```python
from build123d import *

# Parameters (mm, degrees)
BOSS_EXTRUDE1_DEPTH    = 11
SKETCH2_R              = 13
BOSS_EXTRUDE2_DEPTH    = 1
SKETCH3_R              = 9.5
CUT_EXTRUDE1_DEPTH     = 25.372115214
M5_TAPPED_HOLE1_REACH  = 37.623
M5_TAPPED_HOLE1_BORE_R = 2.1
M5_TAPPED_HOLE2_REACH  = 37.623
M5_TAPPED_HOLE2_BORE_R = 2.1


with BuildPart() as part:
    # Sketch1 → Boss-Extrude1 (new body)
    with BuildSketch(Plane.XY):
        with BuildLine():
            Line((-9.013878189, 15), (9.013878189, 15))
            ThreePointArc((9.013878189, 15), (12.374368671, 12.374368671), (15, 9.013878189))
            Line((15, 9.013878189), (15, -9.013878189))
            ThreePointArc((15, -9.013878189), (12.374368671, -12.374368671), (9.013878189, -15))
            Line((9.013878189, -15), (-9.013878189, -15))
            ThreePointArc((-9.013878189, -15), (-12.374368671, -12.374368671), (-15, -9.013878189))
            Line((-15, -9.013878189), (-15, 9.013878189))
            ThreePointArc((-15, 9.013878189), (-12.374368671, 12.374368671), (-9.013878189, 15))
        make_face()
    extrude(amount=BOSS_EXTRUDE1_DEPTH)

    # Sketch2 → Boss-Extrude2 (add)
    with BuildSketch(Plane.XY.offset(11)):
        Circle(SKETCH2_R)
    extrude(amount=BOSS_EXTRUDE2_DEPTH)

    # Sketch3 → Cut-Extrude1 (cut, through all)
    with BuildSketch(Plane.XY.offset(12)):
        Circle(SKETCH3_R)
    extrude(amount=-CUT_EXTRUDE1_DEPTH, mode=Mode.SUBTRACT)

    # M5 Tapped Hole1 bore → M5 Tapped Hole1 (cut, up to next)
    with BuildSketch(Plane.ZY.offset(15), mode=Mode.PRIVATE) as m5_tapped_hole1_sk1:
        with Locations((5.5, 0)):
            Circle(M5_TAPPED_HOLE1_BORE_R)
    m5_tapped_hole1_tool1 = extrude(m5_tapped_hole1_sk1.sketch, amount=-M5_TAPPED_HOLE1_REACH, mode=Mode.PRIVATE) & part.part
    add(m5_tapped_hole1_tool1.solids().sort_by_distance((-15, 0, 5.5))[0], mode=Mode.SUBTRACT)

    # M5 Tapped Hole2 bore → M5 Tapped Hole2 (cut, up to next)
    with BuildSketch(Plane(origin=(0, 15, 0), x_dir=(-1, 0, 0), z_dir=(0, 1, 0)), mode=Mode.PRIVATE) as m5_tapped_hole2_sk1:
        with Locations((0, 5.5)):
            Circle(M5_TAPPED_HOLE2_BORE_R)
    m5_tapped_hole2_tool1 = extrude(m5_tapped_hole2_sk1.sketch, amount=-M5_TAPPED_HOLE2_REACH, mode=Mode.PRIVATE) & part.part
    add(m5_tapped_hole2_tool1.solids().sort_by_distance((0, 15, 5.5))[0], mode=Mode.SUBTRACT)


solid = part.part
```
Here's how the part is built. I have some questions about the finished solid (model axes, mm). A direction names the side the tool comes from. Round coordinates to 2 decimals unless told otherwise and drop trailing zeros. Loops run counter-clockwise (first coordinate to the right, second up) from the corner with the lowest first, then second, coordinate; pieces in that order, holes last.
1. Suppose I cut it at B-B, the plane y = 0. Please give me the cut outline in (x, z).
Answers:
outline: (-15, 0) - (-9.5, 0) - (-9.5, 3.4) - (-15, 3.4) - close; (-15, 7.6) - (-9.5, 7.6) - (-9.5, 12) - (-13, 12) - (-13, 11) - (-15, 11) - close; (9.5, 0) - (15, 0) - (15, 11) - (13, 11) - (13, 12) - (9.5, 12) - close
2. Suppose I cut it at C-C, the plane z = 9.5. Please give me the cut outline in (x, y), and give its area (3 significant figures).
Answers:
outline: (-15, -9.01) arc R17.5 ccw to (-9.01, -15) - (9.01, -15) arc R17.5 ccw to (15, -9.01) - (15, 9.01) arc R17.5 ccw to (9.01, 15) - (-9.01, 15) arc R17.5 ccw to (-15, 9.01) - close; hole circle Ø19 at (0, 0)
area: 557 mm2
3. For faces 4 (the face through (15, 0, 5)), 5 (the face through (-12.173, 0.631, 7.503)), 6 (the face through (-10.316, -7.91, 11.493)), which set-ups out of +Z, -Z, +X, -X, +Y, -Y let a thin tool reach every point of the face, with its end or its side?
Answers:
face 4: +Z, -Z, +X, +Y, -Y
face 5: -X
face 6: +Z
4. If I drill on probe 1 along X at (y, z) = (-3, 2.5); probe 2 along Z at (x, y) = (0, 13.8); probe 3 along Z at (x, y) = (-10, 12), over which ranges is the centre line in solid material (lowest first)?
Answers:
probe 1: x = -15 to -9.01, 9.01 to 15
probe 2: z = 0 to 3.4, 7.6 to 11
probe 3: z = 0 to 11
5. Thinking about a two-plate mould opening in Z: for faces 1 (the face through (7, 7, 0)), 2 (the face through (12.33, 12.42, 5.42)), 3 (the face through (0.273, 12.169, 7.582)), which applies, released by +Z, released by -Z, zero draft, split by the parting line, or undercut?
Answers:
face 1: released by -Z
face 2: zero draft
face 3: undercut
6. Suppose I cut it at A-A, the plane z = 5.5. Please give me the cut outline in (x, y).
Answers:
outline: (-15, -9.01) arc R17.5 ccw to (-9.01, -15) - (9.01, -15) arc R17.5 ccw to (15, -9.01) - (15, 9.01) arc R17.5 ccw to (9.01, 15) - (2.1, 15) - (2.1, 9.26) arc R9.5 cw (long way) to (-9.26, -2.1) - (-15, -2.1) - close; (-15, 2.1) - (-9.26, 2.1) arc R9.5 cw to (-2.1, 9.26) - (-2.1, 15) - (-9.01, 15) arc R17.5 ccw to (-15, 9.01) - close
7. Suppose I cut it at D-D, the plane x = 3. Please give me the cut outline in (y, z), and give its area (3 significant figures).
Answers:
outline: (-15, 0) - (-9.01, 0) - (-9.01, 12) - (-12.65, 12) - (-12.65, 11) - (-15, 11) - close; (9.01, 0) - (15, 0) - (15, 11) - (12.65, 11) - (12.65, 12) - (9.01, 12) - close
area: 139 mm2
8. Will these pins go through, and if not, where does the flat tip stop? pin 1 (1.5 mm diameter, centred on y = 10.5, z = 8, fed in from -X); pin 2 (9 mm diameter, centred on x = 0.5, y = -0.5, fed in from +Z); pin 3 (4 mm diameter, centred on x = 10.5, y = 10.5, fed in from -Z); pin 4 (3.5 mm diameter, centred on y = 0, z = 5.5, fed in from -X).
Answers:
pin 1: stops at x = -14.53
pin 2: passes through
pin 3: stops at z = 0
pin 4: stops at x = 9.34
